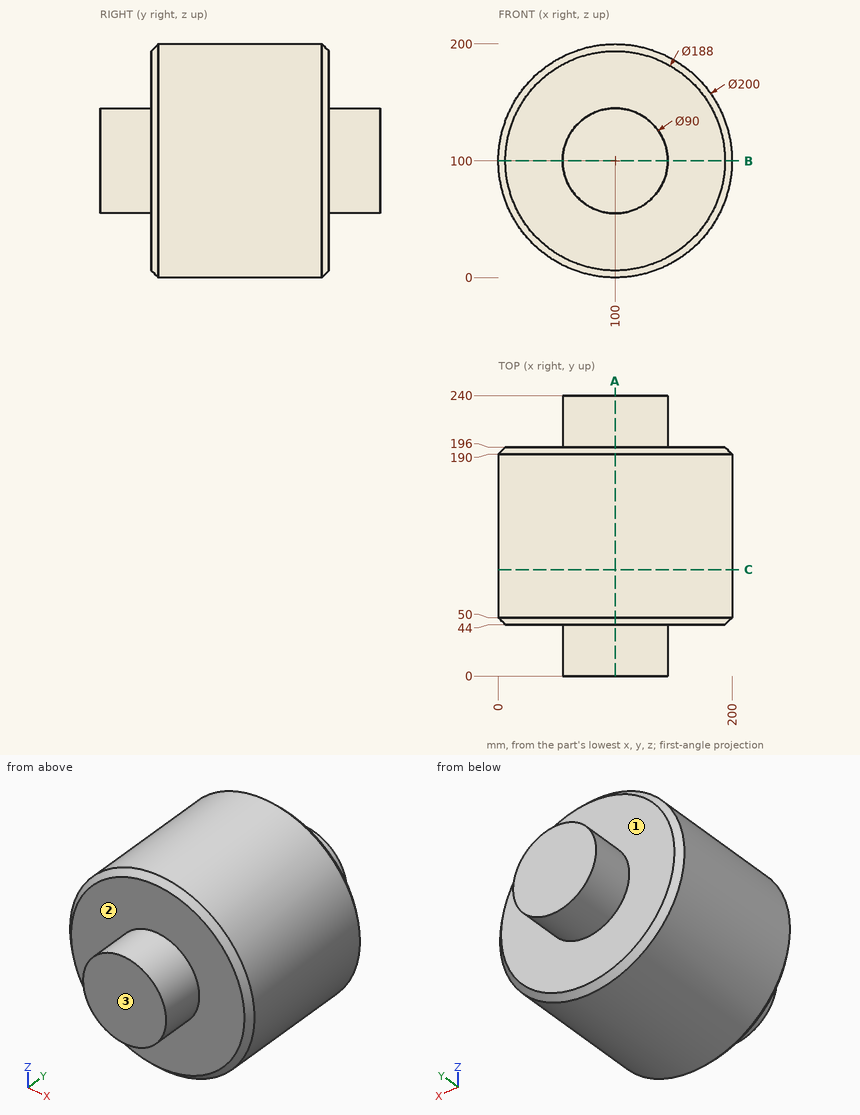
Study the drawing (mm; zero at the part's minimum x, y, z) and answer. A direction names the side the tool comes from. Round coordinates to 2 decimals unless told otherwise and drop trailing zeros. Loops run counter-clockwise (first coordinate to the right, second up) from the corner with the lowest first, then second, coordinate; pieces in that order, holes last. Notation, with made-up numbers: (70, -28.75) -> (119, -28.75) arc R20 cw to (119, 6.25) -> close; hole circle Ø9 at (44.5, 76.25). An arc over 180 degrees is marked (long way). One line per item, written item: value.
1) A cutting plane is placed at C-C (y = 91). Determine the outline of the cut face in (x, z).
Answer list:
outline: circle Ø200 at (100, 100)
2) A cutting plane is placed at B-B (z = 100). Determine the outline of the cut face in (x, y), and give its area (3 significant figures).
Answer list:
outline: (0, 50) -> (6, 44) -> (55, 44) -> (55, 0) -> (145, 0) -> (145, 44) -> (194, 44) -> (200, 50) -> (200, 190) -> (194, 196) -> (145, 196) -> (145, 240) -> (55, 240) -> (55, 196) -> (6, 196) -> (0, 190) -> close
area: 38,200 mm²
3) Flat-ended cylindrical pins translate along their axes: P1, Ø10, axis at x = 80, y = 174, coming from the +Z side; P2, Ø3, axis at y = 165, z = 129.5, coming from the -X side; P3, Ø8, axis at y = 42, z = 76, coming from the -X side. Find the tip coordinate at first contact, or state that the pin passes through.
Answer list:
P1: stops at z = 198.87
P2: stops at x = 4
P3: stops at x = 6.93
4) Consider L1, parallel to Y at x = 112, z = 160.5; L2, parallel to Z at x = 97.5, y = 171; L3, parallel to Z at x = 51, y = 135. Determine where each line is inside the solid, lowest interval first. Write a range as [from, to].
Answer list:
L1: y = [44, 196]
L2: z = [0.03, 199.97]
L3: z = [12.83, 187.17]
5) A cutting plane is placed at A-A (x = 100). Determine the outline of the cut face in (y, z), and give its area (3 significant figures).
Answer list:
outline: (0, 55) -> (44, 55) -> (44, 6) -> (50, 0) -> (190, 0) -> (196, 6) -> (196, 55) -> (240, 55) -> (240, 145) -> (196, 145) -> (196, 194) -> (190, 200) -> (50, 200) -> (44, 194) -> (44, 145) -> (0, 145) -> close
area: 38,200 mm²
6) For the marked faces 1, 2 and 3, determine the directions among +Z, -Z, +X, -X, +Y, -Y from which every point of the face is accessible in a straight line to the end or side of a thin tool.
Answer list:
face 1: +Y
face 2: -Y
face 3: +Z, -Z, +X, -X, -Y
